Model file for the job. Use its own axes, mm. Face numbers are marked on the shaded views. A direction names the side the tool comes from. Round coordinates to 2 decimals unless told otherwise and drop trailing zeros. Loops run counter-clockwise (first coordinate to the right, second up) from the corner with the lowest first, then second, coordinate; pieces in that order, holes last. Notation, with made-up numbers: (-39, -12) -> (-26, -12) arc R17 ccw to (-26, 18) -> close; hole circle Ø1 at (72.5, 74.25). An arc over 180 degrees is marked (long way). Use a Markdown table: item, result. Add a question column.
```python
from build123d import *

# Parameters (mm, degrees)
BOSS_EXTRUDE1_DEPTH = 60
CUT_EXTRUDE1_DEPTH  = 40
BOSS_EXTRUDE2_REACH = 77.842
SKETCH3_R           = 5


with BuildPart() as part:
    # Sketch1 → Boss-Extrude1 (new body)
    with BuildSketch(Plane(origin=(0, 0, 0), x_dir=(1, 0, 0), z_dir=(0, 1, 0))):
        with BuildLine():
            Line((0, 0), (0, -40))
            Line((0, -40), (-32.916811342, -30.326541582))
            ThreePointArc((-32.916811342, -30.326541582), (-40.645313725, -20), (-32.916811342, -9.673458418))
            Line((-32.916811342, -9.673458418), (0, 0))
        make_face()
    extrude(amount=BOSS_EXTRUDE1_DEPTH)

    # Sketch2 → Cut-Extrude1 (cut)
    with BuildSketch(Plane(origin=(0, 10, 0), x_dir=(-1, 0, 0), z_dir=(0, -1, 0))):
        with BuildLine():
            Line((5.381519546, -1.581499041), (5.381519546, -38.418500959))
            Line((5.381519546, -38.418500959), (32.916811342, -30.326541582))
            ThreePointArc((32.916811342, -30.326541582), (40.645313725, -20), (32.916811342, -9.673458418))
            Line((32.916811342, -9.673458418), (5.381519546, -1.581499041))
        make_face()
    extrude(amount=-CUT_EXTRUDE1_DEPTH, mode=Mode.SUBTRACT)

    # Sketch3 → Boss-Extrude2 (add, up to next)
    with BuildSketch(Plane(origin=(0, 10, 0), x_dir=(-1, 0, 0), z_dir=(0, -1, 0)), mode=Mode.PRIVATE) as boss_extrude2_sk1:
        with Locations(Location((29.882089371, -20, 0), (0, 0, 90))):
            Circle(SKETCH3_R)
    boss_extrude2_tool1 = extrude(boss_extrude2_sk1.sketch, amount=-BOSS_EXTRUDE2_REACH, mode=Mode.PRIVATE) - part.part
    add(boss_extrude2_tool1.solids().sort_by_distance((-29.882089, 10, 20))[0])


solid = part.part
```
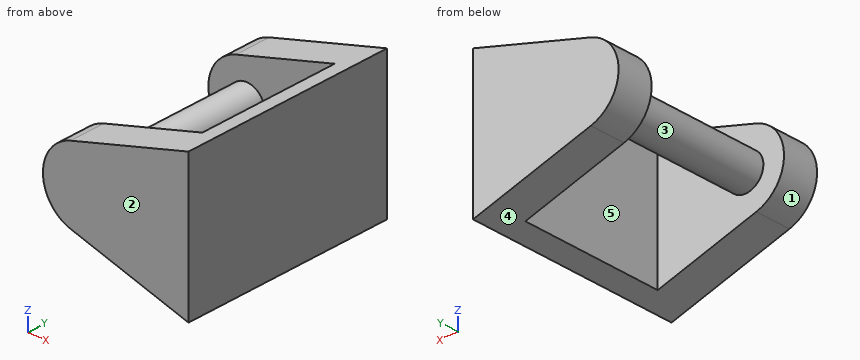
1) Tool access for the marked faces 4 and 5: list every direction of +Z, -Z, +X, -X, +Y, -Y with a clear straight run to the whole face (end or side of a thin tool).
2) Cut at B-B on x = -14. Write the cut outline in (y, z), and give its area (3 significant figures).
3) Wall check: probe 1 along Y at (x, z) = (-8, 3); probe 2 along X at (y, z) = (29.5, 20); probe 3 along X at (y, z) = (34, 5). Give the ranges that are in metal, low to high. Write a range as from..to.
4) Pull direction Y, two halves, no side cores. Call the marked faces 1, 2 and 3: +Y half, -Y half, draft (parallel to the pull), parting line (faces both ways), or undercut.
5) Pin check, flat tips, straight feed: pin 1 Ø1 at (y, z) = (21.5, 9.5) entering from -X; pin 2 Ø11 at (y, z) = (27, 16) entering from -X. Stop position of each tip, or through.
6) Cut at D-D on z = 37. Write the cut outline in (x, y).
7) Cut at A-A on z = 20. Write the cut outline in (x, y).
8) Cut at C-C on y = 40.5. Write the cut outline in (x, z), and give its area (3 significant figures).
Established:
| question | item | result |
|---|---|---|
| 1 | face 4 | -Z, -X, +Y, -Y |
| 1 | face 5 | +Z, -Z |
| 2 | outline | (0, 4.11) -> (10, 4.11) -> (10, 35.89) -> (0, 35.89) -> close; (50, 4.11) -> (60, 4.11) -> (60, 35.89) -> (50, 35.89) -> close |
| 2 | area | 635 mm^2 |
| 3 | probe 1 | y = 0..10, 50..60 |
| 3 | probe 2 | x = -34.88..-24.88, -5.38..0 |
| 3 | probe 3 | x = -5.38..0 |
| 4 | face 1 | draft |
| 4 | face 2 | -Y half |
| 4 | face 3 | undercut |
| 5 | pin 1 | stops at x = -5.38 |
| 5 | pin 2 | stops at x = -34.88 |
| 6 | outline | (-10.21, 0) -> (0, 0) -> (0, 60) -> (-10.21, 60) -> (-10.21, 50) -> (-5.38, 50) -> (-5.38, 10) -> (-10.21, 10) -> close |
| 7 | outline | (-40.65, 0) -> (0, 0) -> (0, 60) -> (-40.65, 60) -> (-40.65, 50) -> (-34.88, 50) -> (-34.88, 10) -> (-40.65, 10) -> close; hole (-24.88, 10) -> (-5.38, 10) -> (-5.38, 50) -> (-24.88, 50) -> close |
| 8 | outline | circle Ø10 at (-29.88, 20); (-5.38, 1.58) -> (0, 0) -> (0, 40) -> (-5.38, 38.42) -> close |
| 8 | area | 285 mm^2 |
